from build123d import *

# Parameters (mm, degrees)
SKETCH1_R   = 2.5
SKETCH1_R_2 = 2


with BuildPart() as part:
    # Sweep1: sweep along a path in Sketch2
    with BuildLine(Plane(origin=(0, 0, 0), x_dir=(1, 0, 0), z_dir=(0, 1, 0))) as sweep1_path:
        Line((0, 0), (0, -20))
        ThreePointArc((0, -20), (-1.464466094, -23.535533906), (-5, -25))
        Line((-5, -25), (-30, -25))
    # Sketch1 → Sweep1 (sweep)
    with BuildSketch(Plane.XY):
        Circle(SKETCH1_R)
        Circle(SKETCH1_R_2, mode=Mode.SUBTRACT)
    sweep(path=sweep1_path.line)


solid = part.part
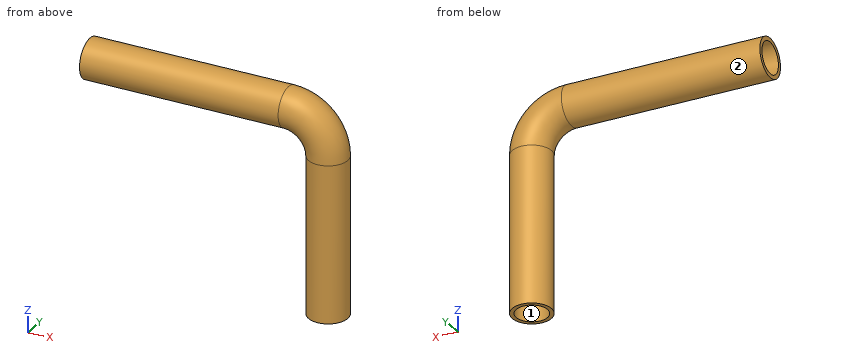
Read the model definition and answer for the solid it produces. Units are mm, in the model's axes. Face numbers are marked on the shaded views. Round coordinates to 2 decimals unless told otherwise and drop trailing zeros. Write each loop counter-clockwise with the first axis right and the second up, starting at its lowest first coordinate (ties: lowest second). Pieces come first, ordered by that corner, then holes.
1. Straight lines are drawn through the part: L1, parallel to Z at x = -20, y = 0; L2, parallel to Y at x = 0, z = 12.75; L3, parallel to Z at x = -16, y = -1.6. For each, find the intervals that lie inside material, in ascending order.
2. Given pin 1 Ø1.5 at (y, z) = (0, 7) entering from -X; pin 2 Ø1 at (y, z) = (-2, 14.5) entering from -X; pin 3 Ø5 at (x, z) = (-11.5, 23.5) entering from -Y, each flat-ended and moving along its own axis, determine where each tip first touches the part or whether it passes through.
3. Determine the mould class of the marked faces 1 and 2 for opening direction Y: pulls with the +Y half, pulls with the -Y half, needs draft (parallel to the pull), parting line crosses it, or undercut.
4. The part is cut by section A-A, the plane y = 0. Determine the outline of the cut face in (x, z), then the cut area to 3 significant figures.
5. The part is cut by section D-D, the plane y = -1.55. Determine the outline of the cut face in (x, z).
6. The part is cut by section B-B, the plane x = -11.5. Determine the outline of the cut face in (y, z).
7. The part is cut by section C-C, the plane z = 8.5. Determine the outline of the cut face in (x, y).
Values:
1. L1: z = 22.5 to 23, 27 to 27.5
1. L2: y = -2.5 to -2, 2 to 2.5
1. L3: z = 23.08 to 23.8, 26.2 to 26.92
2. pin 1: stops at x = -2.5
2. pin 2: stops at x = -2
2. pin 3: stops at y = -2.5
3. face 1: undercut
3. face 2: parting line crosses it
4. outline: (-30, 22.5) - (-5, 22.5) arc R2.5 cw to (-2.5, 20) - (-2.5, 0) - (-2, 0) - (-2, 20) arc R3 ccw to (-5, 23) - (-30, 23) - close; (-30, 27) - (-5, 27) arc R7 cw to (2, 20) - (2, 0) - (2.5, 0) - (2.5, 20) arc R7.5 ccw to (-5, 27.5) - (-30, 27.5) - close
4. area: 52.9 mm2
5. outline: (-30, 23.04) - (-5, 23.04) arc R3.04 cw to (-1.96, 20) - (-1.96, 0) - (-1.26, 0) - (-1.26, 20) arc R3.74 ccw to (-5, 23.74) - (-30, 23.74) - close; (-30, 26.26) - (-5, 26.26) arc R6.26 cw to (1.26, 20) - (1.26, 0) - (1.96, 0) - (1.96, 20) arc R6.96 ccw to (-5, 26.96) - (-30, 26.96) - close
6. outline: circle Ø5 at (0, 25); hole circle Ø4 at (0, 25)
7. outline: circle Ø5 at (0, 0); hole circle Ø4 at (0, 0)
